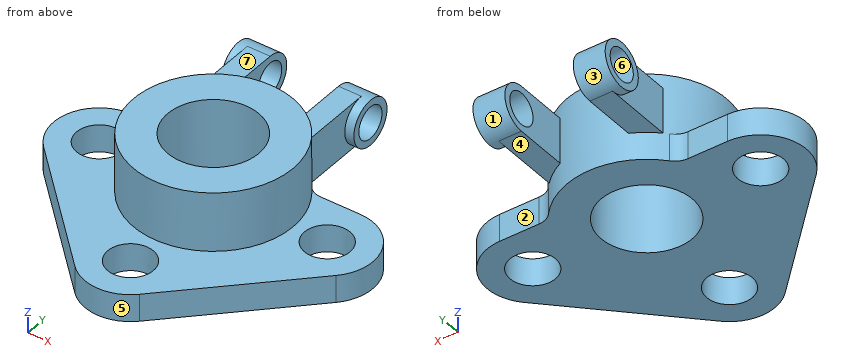
```python
from build123d import *
from build123d.topology import SkipClean

# Parameters (mm, degrees)
HUB_PROFILE_SKETCH_R     = 35
HUB_PROFILE_SKETCH_R_2   = 20
HUB_70_BORE_40_DEPTH     = 38
MOUNTING_FLANGE_SKETCH_R = 10
MOUNTING_FLANGE_DEPTH    = 12
FLANGE_HUB_FILLET_R8_R   = 8
CLEVIS_LUG_SKETCH_W      = 10
CLEVIS_LUG_SKETCH_H      = 20
CLEVIS_LUGS_DEPTH        = 32
LUG_BOSS_SKETCH_A_R      = 10
LUG_BOSS_SKETCH_A_R_2    = 7
LUG_BOSS_A_20_DEPTH      = 14
PIN_START                = -50
PIN_HOLE_SKETCH_R        = 7
PIN_HOLE_14_DEPTH        = 50
LUG_START                = -14
LUG_BOSS_SKETCH_B_R      = 10
LUG_BOSS_SKETCH_B_R_2    = 7
LUG_BOSS_B_20_DEPTH      = 14


with BuildPart() as part:
    # Hub Profile Sketch → Hub Ø70 Bore Ø40 (new body)
    with BuildSketch(Plane.XY):
        Circle(HUB_PROFILE_SKETCH_R)
        Circle(HUB_PROFILE_SKETCH_R_2, mode=Mode.SUBTRACT)
    extrude(amount=HUB_70_BORE_40_DEPTH)

    # Mounting Flange Sketch → Mounting Flange (add)
    with BuildSketch(Plane.XY):
        with BuildLine():
            Line((50, 20), (28.722813233, 20))
            ThreePointArc((28.722813233, 20), (0, -35), (-28.722813233, 20))
            Line((-28.722813233, 20), (-50, 20))
            ThreePointArc((-50, 20), (-68.47759065, 7.653668647), (-64.142135624, -14.142135624))
            Line((-64.142135624, -14.142135624), (-14.142135624, -64.142135624))
            ThreePointArc((-14.142135624, -64.142135624), (0, -70), (14.142135624, -64.142135624))
            Line((14.142135624, -64.142135624), (64.142135624, -14.142135624))
            ThreePointArc((64.142135624, -14.142135624), (68.47759065, 7.653668647), (50, 20))
        make_face()
        with Locations((50, 0)):
            Circle(MOUNTING_FLANGE_SKETCH_R, mode=Mode.SUBTRACT)
        with Locations((0, -50)):
            Circle(MOUNTING_FLANGE_SKETCH_R, mode=Mode.SUBTRACT)
        with Locations(Location((-50, 0, 0), (0, 0, 180))):
            Circle(MOUNTING_FLANGE_SKETCH_R, mode=Mode.SUBTRACT)
    extrude(amount=MOUNTING_FLANGE_DEPTH)

    # Flange Hub Fillet R8
    flange_hub_fillet_r8_edges = [part.edges().sort_by_distance(p)[0] for p in [
        (28.722813233, 20, 6),
        (-28.722813233, 20, 6),
    ]]
    fillet(flange_hub_fillet_r8_edges, radius=FLANGE_HUB_FILLET_R8_R)

    # Clevis Lug Sketch → Clevis Lugs (add)
    with BuildSketch(Plane(origin=(0, 55, 0), x_dir=(1, 0, 0), z_dir=(0, 1, 0))):
        with Locations((-20, -22)):
            Rectangle(CLEVIS_LUG_SKETCH_W, CLEVIS_LUG_SKETCH_H)
        with Locations((20, -22)):
            Rectangle(CLEVIS_LUG_SKETCH_W, CLEVIS_LUG_SKETCH_H)
    extrude(amount=-CLEVIS_LUGS_DEPTH)

    # Lug Boss Sketch A → Lug Boss A Ø20 (add)
    with BuildSketch(Plane.ZY.offset(-15)):
        with Locations((22, 55)):
            Circle(LUG_BOSS_SKETCH_A_R)
        with Locations((22, 55)):
            Circle(LUG_BOSS_SKETCH_A_R_2, mode=Mode.SUBTRACT)
    extrude(amount=-LUG_BOSS_A_20_DEPTH)

    # Pin Hole Sketch → Pin Hole Ø14 (cut)
    with SkipClean():  # the faces are left unmerged after this step: merging them gives an invalid solid
        with BuildSketch(Plane(origin=(25, 0, 0), x_dir=(0, 0, -1), z_dir=(1, 0, 0)).offset(PIN_START)):
            with Locations(Location((-22, 55, 0), (0, 0, 180))):
                Circle(PIN_HOLE_SKETCH_R)
        extrude(amount=PIN_HOLE_14_DEPTH, mode=Mode.SUBTRACT)

    # Lug Boss Sketch B → Lug Boss B Ø20 (add)
    with SkipClean():  # the faces are left unmerged after this step: merging them gives an invalid solid
        with BuildSketch(Plane(origin=(-15, 0, 0), x_dir=(0, 0, -1), z_dir=(1, 0, 0)).offset(LUG_START)):
            with Locations(Location((-22, 55, 0), (0, 0, 180))):
                Circle(LUG_BOSS_SKETCH_B_R)
            with Locations(Location((-22, 55, 0), (0, 0, 180))):
                Circle(LUG_BOSS_SKETCH_B_R_2, mode=Mode.SUBTRACT)
        extrude(amount=LUG_BOSS_B_20_DEPTH)


solid = part.part
```
Part model, mm, in its own coordinate system. Face numbers are marked on the shaded views. A direction names the side the tool comes from. Give positions to 0.01 mm unless a question says otherwise; leave off trailing zeros. Loops run counter-clockwise (first coordinate to the right, second up) from the corner with the lowest first, then second, coordinate; pieces in that order, holes last. Notation, with made-up numbers: M 11.25,8.25 L 67.25,8.25 A15 cw 67.25,13.25 Z; hole C 80.5,23 d3. An arc over 180 degrees is marked long. Return JSON: item names as keys, results as strings.
1) Pull direction Y, two halves, no side cores. Call the marked faces 5, 6 and 7: released by +Y, released by -Y, zero draft, split by the parting line, or undercut.
Calculated:
{"face 5": "released by -Y", "face 6": "undercut", "face 7": "zero draft"}
2) Saw through at D-D, the plane z = 4.5. List the corners of the cut face in (x, y), then the cut area to 3 significant figures.
Calculated:
{"outline": "M -64.14,-14.14 L -14.14,-64.14 A20 ccw 14.14,-64.14 L 64.14,-14.14 A20 ccw 50,20 L 32.63,20 A8 cw 26.56,22.79 A35 ccw -26.56,22.79 A8 cw -32.63,20 L -50,20 A20 ccw Z; hole C -50,0 d20; hole C 0,0 d40; hole C 0,-50 d20; hole C 50,0 d20", "area": "6,990 mm2"}
3) Saw through at A-A, the plane z = 22. List the corners of the cut face in (x, y), then the cut area to 3 significant figures.
Calculated:
{"outline": "M -29,45 L -25,45 L -25,24.49 A35 ccw long 25,24.49 L 25,45 L 29,45 L 29,48 L 15,48 L 15,31.62 A35 ccw -15,31.62 L -15,48 L -29,48 Z; M -29,62 L -15,62 L -15,65 L -29,65 Z; M 15,62 L 29,62 L 29,65 L 15,65 Z; hole C 0,0 d40", "area": "3,090 mm2"}
4) 3-axis set-ups, long thin cutter, end or side, ignore diameter. For the marked faces 1, 2, 3 and 4: which of +Z, -Z, +X, -X, +Y, -Y reach the whole face in a straight line?
Calculated:
{"face 1": "+X", "face 2": "+Z, -Z, +X, +Y", "face 3": "-X", "face 4": "-Z, +X, +Y"}
5) Flat gauge pins, fed straight in: pin 1 Ø2 at (x, z) = (-25.5, 8.5) entering from +Y (3 decimals); pin 2 Ø6 at (y, z) = (47, 20) entering from +X; pin 3 Ø9.5 at (x, z) = (45, 3) entering from +Y; pin 4 Ø6 at (y, z) = (56.5, 24) entering from -X (1 decimal). Where does each tip first touch, or does it go through?
Calculated:
{"pin 1": "stops at y = 24.995", "pin 2": "stops at x = 29", "pin 3": "stops at y = 20", "pin 4": "passes through"}
6) Saw through at B-B, the plane y = 0. List the corners of the cut face in (x, z), then the cut area to 3 significant figures.
Calculated:
{"outline": "M -70,0 L -60,0 L -60,12 L -70,12 Z; M -40,0 L -20,0 L -20,38 L -35,38 L -35,12 L -40,12 Z; M 20,0 L 40,0 L 40,12 L 35,12 L 35,38 L 20,38 Z; M 60,0 L 70,0 L 70,12 L 60,12 Z", "area": "1,500 mm2"}
7) Saw through at C-C, the plane y = -43.5. List the corners of the cut face in (x, z).
Calculated:
{"outline": "M -34.78,0 L -7.6,0 L -7.6,12 L -34.78,12 Z; M 7.6,0 L 34.78,0 L 34.78,12 L 7.6,12 Z"}
8) Drill centre lines: line 1 (X direction, y = 53, z = 12.5); line 2 (Y direction, x = -2.5, z = 2.5); line 3 (X direction, y = -1, z = 13). Where is each one in solid material? Low to high.
Calculated:
{"line 1": "x = -29 to -15, 15 to 29", "line 2": "y = -69.84 to -59.68, -40.32 to -19.84, 19.84 to 34.91", "line 3": "x = -34.99 to -19.97, 19.97 to 34.99"}
